Geometry check sheet. Reference: the model listing, model coordinates, mm. Face numbers are marked on the shaded views. A direction names the side the tool comes from. Round coordinates to 2 decimals unless told otherwise and drop trailing zeros. Write each loop counter-clockwise with the first axis right and the second up, starting at its lowest first coordinate (ties: lowest second). Pieces come first, ordered by that corner, then holes. Notation, with made-up numbers: (-28.75, 37) - (-2.75, 37) arc R21 ccw to (-2.75, 56) - close; hole circle Ø8 at (-28.75, -16.75). An arc over 180 degrees is marked (long way). Return JSON: item names as keys, results as strings. Group by question number.
from build123d import *

# Parameters (mm, degrees)
BOSS_EXTRUDE1_DEPTH        = 20
MOVE_FACE1_BY              = 3.4
MOVE_FACE2_BY              = 9.9
BOSS_EXTRUDE2_DEPTH        = 20
M3_TAPPED_HOLE1_D          = 2.5
M3_TAPPED_HOLE1_DEPTH      = 10
M3_TAPPED_HOLE1_TIP        = 0.751075774
SKETCH13_W                 = 4
SKETCH13_H                 = 8
BOSS_EXTRUDE3_DEPTH        = 9.9
M3_TAPPED_HOLE2_D          = 2.5
M3_TAPPED_HOLE2_DEPTH      = 10
M3_TAPPED_HOLE2_TIP        = 0.751075774
CHAMFER1_SIZE              = 1
SIZE_MM_DOWEL_HOLE_0_D     = 1.5
SIZE_MM_DOWEL_HOLE_0_DEPTH = 6
SIZE_MM_DOWEL_HOLE_0_TIP   = 0.450645464


with BuildPart() as part:
    # Sketch1 → Boss-Extrude1 (new body)
    with BuildSketch(Plane.XY):
        with BuildLine():
            Line((0, 0), (0, 6.5))
            Line((0, 6.5), (4.9, 6.5))
            Line((4.9, 6.5), (4.9, 4.058257569))
            ThreePointArc((4.9, 4.058257569), (4.746446609, 3.246446609), (5.558257569, 3.4))
            Line((5.558257569, 3.4), (8, 3.4))
            Line((8, 3.4), (8, 0))
            Line((8, 0), (0, 0))
        make_face()
    extrude(amount=BOSS_EXTRUDE1_DEPTH)

    # Move Face1: a face moved outward by 3.4
    extrude(part.faces().sort_by_distance((2.45, 6.5, 10))[0], amount=MOVE_FACE1_BY, dir=(0, 1, 0))

    # Move Face2: a face moved outward by 9.9
    extrude(part.faces().sort_by_distance((8, 1.7, 10))[0], amount=MOVE_FACE2_BY, dir=(1, 0, 0))

    # Sketch10 → Boss-Extrude2 (add)
    with BuildSketch(Plane(origin=(0, 0, 0), x_dir=(-1, 0, 0), z_dir=(0, 0, -1))):
        Polygon((-17.9, 3.4), (-17.9, 4.9), (-14.4, 4.9), (-12.9, 3.4), align=None)
    extrude(amount=-BOSS_EXTRUDE2_DEPTH)

    # M3 Tapped Hole1
    with Locations(Plane(origin=(0, 0, 0), x_dir=(-1, 0, 0), z_dir=(0, -1, 0))):
        with Locations((-13.9, -10)):
            Hole(M3_TAPPED_HOLE1_D / 2, depth=M3_TAPPED_HOLE1_DEPTH)
            with Locations((0, 0, -(M3_TAPPED_HOLE1_DEPTH + M3_TAPPED_HOLE1_TIP / 2))):  # 118° drill point
                Cone(0, M3_TAPPED_HOLE1_D / 2, M3_TAPPED_HOLE1_TIP, mode=Mode.SUBTRACT)

    # Sketch13 → Boss-Extrude3 (add)
    with BuildSketch(Plane.XZ):
        with Locations((-2, 4)):
            Rectangle(SKETCH13_W, SKETCH13_H)
    extrude(amount=-BOSS_EXTRUDE3_DEPTH)

    # M3 Tapped Hole2
    with Locations(Plane(origin=(0, 0, 0), x_dir=(-1, 0, 0), z_dir=(0, -1, 0))):
        with Locations((-13.45, -16), (0.55, -4)):
            Hole(M3_TAPPED_HOLE2_D / 2, depth=M3_TAPPED_HOLE2_DEPTH)
            with Locations((0, 0, -(M3_TAPPED_HOLE2_DEPTH + M3_TAPPED_HOLE2_TIP / 2))):  # 118° drill point
                Cone(0, M3_TAPPED_HOLE2_D / 2, M3_TAPPED_HOLE2_TIP, mode=Mode.SUBTRACT)

    # Chamfer1
    chamfer1_edges = [part.edges().sort_by_distance(p)[0] for p in [
        (0, 4.95, 20),
        (-4, 4.95, 0),
        (-4, 4.95, 8),
        (17.9, 2.45, 20),
        (17.9, 2.45, 0),
    ]]
    chamfer(chamfer1_edges, length=CHAMFER1_SIZE)

    # Size mm dowel hole 0
    with Locations(Plane(origin=(17.9, 0, 0), x_dir=(0, 0, -1), z_dir=(1, 0, 0))):
        with Locations((-5, 1.75)):
            Hole(SIZE_MM_DOWEL_HOLE_0_D / 2, depth=SIZE_MM_DOWEL_HOLE_0_DEPTH)
            with Locations((0, 0, -(SIZE_MM_DOWEL_HOLE_0_DEPTH + SIZE_MM_DOWEL_HOLE_0_TIP / 2))):  # 118° drill point
                Cone(0, SIZE_MM_DOWEL_HOLE_0_D / 2, SIZE_MM_DOWEL_HOLE_0_TIP, mode=Mode.SUBTRACT)


solid = part.part
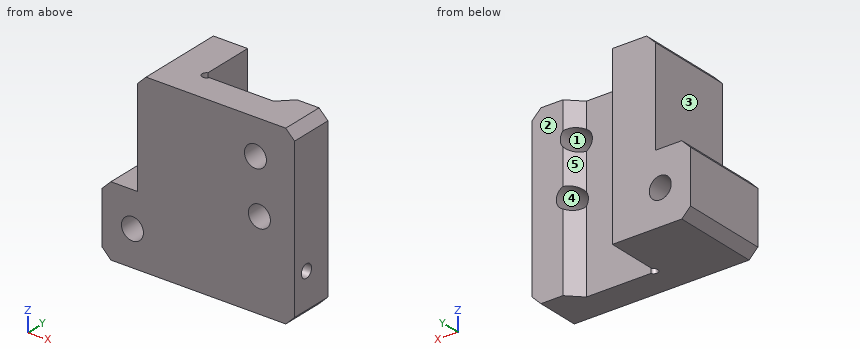
1. Mould release check, pull along X, two halves, no side actions. Record for the marked faces 1, 2 and 3: pulls with the +X half, pulls with the -X half, needs draft (parallel to the pull), parting line crosses it, or undercut.
2. Section check A-A (x = 13.9). Enter the section's corners in (y, z), and give its area (3 significant figures).
3. Material ranges on line 1 along Z through (x, y) = (14.9, 1.75); line 2 along X through (y, z) = (1.35, 16); line 3 along Z through (x, y) = (-0.55, 2), recorded low to high.
4. Tool access check on the marked faces 4 and 5. Record the directions out of +Z, -Z, +X, -X, +Y, -Y that give a thin tool (end or side, any length) a straight path to the whole face; none if there is none.
5. Section check B-B (z = 10). Enter the section's corners in (x, y), and give its area (3 significant figures).
6. Depth check by flat-ended pin: pin 1 Ø5 at (x, z) = (6.5, 7.5) entering from -Y; pin 2 Ø1 at (y, z) = (8, 16.5) entering from -X; pin 3 Ø2 at (x, z) = (10, 9) entering from +Y; pin 4 Ø1 at (x, z) = (16, 5.5) entering from +Y. Enter the tip coordinate at first touch or a pass-through.
7. Section check C-C (x = 16.25). Enter the section's corners in (y, z).
8. Section check D-D (y = 6.5). Enter the section's corners in (x, z).
Result sheet:
{
 "1": {"face 1": "undercut", "face 2": "needs draft", "face 3": "pulls with the -X half"},
 "2": {"outline": "(0, 0) - (4.4, 0) - (4.4, 8.75) - (0, 8.75) - close; (0, 11.25) - (4.4, 11.25) - (4.4, 14.83) - (0, 14.83) - close; (0, 17.17) - (4.4, 17.17) - (4.4, 20) - (0, 20) - close; hole circle Ø1.5 at (1.75, 5)", "area": "65.0 mm²"},
 "3": {"line 1": "z = 0 to 4.25, 5.75 to 9.25, 10.75 to 20", "line 2": "x = 0 to 12.2, 14.7 to 17.9", "line 3": "z = 0 to 2.75, 5.25 to 8"},
 "4": {"face 4": "+Y, -Y", "face 5": "+Z, -Z, +Y"},
 "5": {"outline": "(0, 0) - (12.65, 0) - (12.65, 3.4) - (5.56, 3.4) arc R0.5 cw (long way) to (4.9, 4.06) - (4.9, 9.9) - (0, 9.9) - close; (15.15, 0) - (17.9, 0) - (17.9, 4.9) - (15.15, 4.9) - close", "area": "88.0 mm²"},
 "6": {"pin 1": "stops at y = 0", "pin 2": "stops at x = 0", "pin 3": "stops at y = 3.4", "pin 4": "stops at y = 4.9"},
 "7": {"outline": "(0, 0) - (4.9, 0) - (4.9, 20) - (0, 20) - close; hole circle Ø1.5 at (1.75, 5)"},
 "8": {"outline": "(-4, 1) - (-3, 0) - (4.9, 0) - (4.9, 20) - (1, 20) - (0, 19) - (0, 8) - (-3, 8) - (-4, 7) - close; hole circle Ø2.5 at (-0.55, 4)"}
}
